from build123d import *

# Parameters (mm, degrees)
SKETCH1_R                  = 15.75
SKETCH1_R_2                = 9.5
BOSS_EXTRUDE1_DEPTH        = 4
SKETCH3_R                  = 10.639095477
SKETCH3_R_2                = 8.5
BOSS_EXTRUDE2_DEPTH        = 2
F_3_1_3_1_DIAMETER_HOLE1_D = 3.1
SKETCH7_R                  = 18.245705154
SKETCH7_R_2                = 13.25
CUT_EXTRUDE1_DEPTH         = 0.45
CHAMFER1_SIZE              = 0.5
CHAMFER2_SIZE              = 0.1


with BuildPart() as part:
    # Sketch1 → Boss-Extrude1 (new, symmetric)
    with BuildSketch(Plane.XY):
        Circle(SKETCH1_R)
        Circle(SKETCH1_R_2, mode=Mode.SUBTRACT)
    extrude(amount=BOSS_EXTRUDE1_DEPTH, both=True)

    # Sketch3 → Boss-Extrude2 (add)
    with BuildSketch(Plane(origin=(0, 0, -4), x_dir=(-1, 0, 0), z_dir=(0, 0, -1))):
        Circle(SKETCH3_R)
        Circle(SKETCH3_R_2, mode=Mode.SUBTRACT)
    extrude(amount=-BOSS_EXTRUDE2_DEPTH)

    # Ø3.1 (3.1) Diameter Hole1 (through all)
    with Locations(Plane(origin=(0, 0, -4), x_dir=(-1, 0, 0), z_dir=(0, 0, -1))):
        with Locations((7.341654592, 8.851559628)):
            f_3_1_3_1_diameter_hole1 = Hole(F_3_1_3_1_DIAMETER_HOLE1_D / 2)

    # Mirror1: Ø3.1 (3.1) Diameter Hole1 across plane
    add(f_3_1_3_1_diameter_hole1.mirror(Plane.ZX), mode=Mode.SUBTRACT)

    # Sketch7 → Cut-Extrude1 (cut)
    with BuildSketch(Plane.XY.offset(4)):
        Circle(SKETCH7_R)
        Circle(SKETCH7_R_2, mode=Mode.SUBTRACT)
    extrude(amount=-CUT_EXTRUDE1_DEPTH, mode=Mode.SUBTRACT)

    # Chamfer1
    chamfer1_edges = [part.edges().sort_by_distance(p)[0] for p in [
        (-15.75, 0, -4),
    ]]
    chamfer(chamfer1_edges, length=CHAMFER1_SIZE)

    # Chamfer2
    chamfer2_edges = [part.edges().sort_by_distance(p)[0] for p in [
        (-9.5, 0, 4),
    ]]
    chamfer(chamfer2_edges, length=CHAMFER2_SIZE)


solid = part.part
Source: CAD feature listing. Evaluate the final solid. Frame: model axes, mm. A direction names the side the tool comes from. Give positions to 0.01 mm unless a question says otherwise; leave off trailing zeros. Order: outer loops, then holes, each group sorted by start corner. A loop starts at its lowest first (then second) coordinate and runs counter-clockwise, first axis right, second up. Notation, with made-up numbers: (63, -14) -> (77, -14) arc R8 cw to (77, -7) -> close; hole circle Ø5 at (-38, 22.5). An arc over 180 degrees is marked (long way). Write item = value, one per line.
Q1. Cut plane C-C, the plane z = -1. Output: boundary loops of the cut face in (x, y), and give its area (3 significant figures).
Data:
outline = circle Ø31.5 at (0, 0); hole circle Ø19 at (0, 0); hole circle Ø3.1 at (-7.34, -8.85); hole circle Ø3.1 at (-7.34, 8.85)
area = 481 mm^2
Q2. Pull-direction query (X, two-part tool) for faces 1 (the face through (-4.57, 7.167, -3.014)), 2 (the face through (6, -8, 4)), 3 (the face through (7.123, 11.172, 3.778)); classes: released by +X, released by -X, zero draft, split by the parting line, or undercut.
Data:
face_1 = undercut
face_2 = zero draft
face_3 = split by the parting line
Q3. Set-up query: faces 4 (the face through (4.38, -8.43, 0.91)), 5 (the face through (-2.05, 15.616, 0.074)). Return all of +Z, -Z, +X, -X, +Y, -Y with unobstructed straight access to the full face (end or side cutting, diameter ignored); none if empty.
Data:
face_4 = +Z
face_5 = +Z, -Z
Q4. Cut plane A-A, the plane y = 0. Output: boundary loops of the cut face in (x, z).
Data:
outline = (-15.75, -3.5) -> (-15.25, -4) -> (-8.5, -4) -> (-8.5, -2) -> (-9.5, -2) -> (-9.5, 3.9) -> (-9.6, 4) -> (-13.25, 4) -> (-13.25, 3.55) -> (-15.75, 3.55) -> close; (8.5, -4) -> (15.25, -4) -> (15.75, -3.5) -> (15.75, 3.55) -> (13.25, 3.55) -> (13.25, 4) -> (9.6, 4) -> (9.5, 3.9) -> (9.5, -2) -> (8.5, -2) -> close
Q5. Material intervals for line 1 (X direction, y = -8.5, z = 2); line 2 (Y direction, x = 0, z = -2.8); line 3 (X direction, y = 8, z = 2.75), sorted ascending. Write a range as from..to.
Data:
line_1 = -13.26..-8.85, -5.83..-4.24, 4.24..13.26
line_2 = -15.75..-8.5, 8.5..15.75
line_3 = -13.57..-8.64, -6.05..-5.12, 5.12..13.57
Q6. Pin query (flat end, axial travel): pin 1 (9.5 mm diameter, centred on x = 4.5, y = -0.5, fed in from +Z); pin 2 (4 mm diameter, centred on x = -8, y = -8.5, fed in from +Z). Return the tip coordinate at first contact, or that it passes through.
Data:
pin_1 = -2
pin_2 = 4
